Check sheet for the modelled part. Datum: model origin and axes. Units: mm. Face numbers are marked on the shaded views. A direction names the side the tool comes from. Round coordinates to 2 decimals unless told otherwise and drop trailing zeros. Order: outer loops, then holes, each group sorted by start corner. A loop starts at its lowest first (then second) coordinate and runs counter-clockwise, first axis right, second up. Notation, with made-up numbers: (24.5, 9) -> (73.5, 9) arc R28 cw to (73.5, 36) -> close; hole circle Ø9 at (24, 10.25). An arc over 180 degrees is marked (long way). Use CSV: the item, a comma, the result in double quotes.
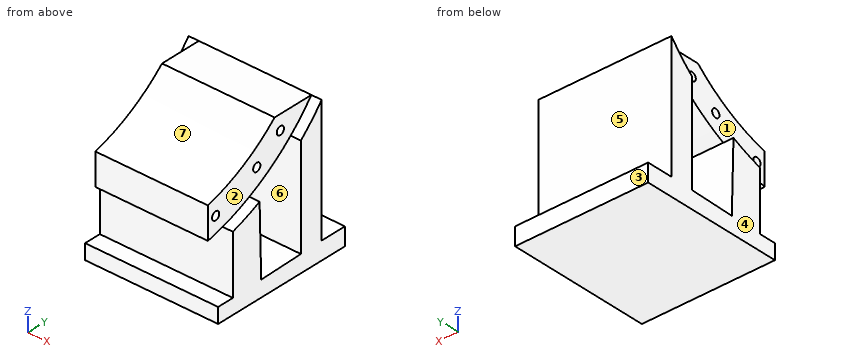
```python
from build123d import *

# Parameters (mm, degrees)
SKETCH1_W               = 130
SKETCH1_H               = 140
BOSS_EXTRUDE1_DEPTH     = 10
SKETCH14_W              = 130
SKETCH14_H              = 140
BOSS_EXTRUDE2_DEPTH     = 130
CUT_EXTRUDE2_DEPTH      = 299.998327755
CUT_EXTRUDE2_DEPTH_BACK = 299.998327755
SKETCH15_W              = 122.59192481
SKETCH15_H              = 25.689880701
CUT_EXTRUDE4_DEPTH      = 299.998327755
CUT_EXTRUDE4_DEPTH_BACK = 10
CUT_EXTRUDE5_DEPTH      = 10
CUT_EXTRUDE6_DEPTH      = 295.78805946
CUT_EXTRUDE6_DEPTH_BACK = 295.78805946
SKETCH19_R              = 4


with BuildPart() as part:
    # Sketch1 → Boss-Extrude1 (new body)
    with BuildSketch(Plane.XY):
        with Locations((65, 160)):
            Rectangle(SKETCH1_W, SKETCH1_H)
    extrude(amount=BOSS_EXTRUDE1_DEPTH)

    # Sketch14 → Boss-Extrude2 (add)
    with BuildSketch(Plane.XY.offset(10)):
        with Locations((65, 160)):
            Rectangle(SKETCH14_W, SKETCH14_H)
    extrude(amount=BOSS_EXTRUDE2_DEPTH)

    # Sketch15 → Cut-Extrude2 (cut, two sides: drawn at the far end of the back side and taken through both)
    with BuildSketch(Plane(origin=(130, 0, 0), x_dir=(0, 0, -1), z_dir=(1, 0, 0)).offset(-CUT_EXTRUDE2_DEPTH_BACK)):
        with BuildLine():
            Line((-140, 90), (-140, 163.652960017))
            ThreePointArc((-140, 163.652960017), (-114.94393992, 129.358801446), (-98.982103949, 90))
            Line((-98.982103949, 90), (-140, 90))
        make_face()
        with BuildLine():
            Line((-68.08230106, 90), (-14.839979069, 90))
            Line((-14.839979069, 90), (-14.839979069, 106.264255909))
            Line((-14.839979069, 106.264255909), (-72.486347105, 106.264255909))
            ThreePointArc((-72.486347105, 106.264255909), (-70.115745067, 98.177775893), (-68.08230106, 90))
        make_face()
        with Locations((-78.704037595, 217.15505965)):
            Rectangle(SKETCH15_W, SKETCH15_H)
        with BuildLine():
            Line((-16.807794328, 181.392341835), (-15.660073853, 137.574182571))
            Line((-15.660073853, 137.574182571), (-84.418578186, 135.773204516))
            ThreePointArc((-84.418578186, 135.773204516), (-98.429747838, 159.645053575), (-115.553810025, 181.392341835))
            Line((-115.553810025, 181.392341835), (-16.807794328, 181.392341835))
        make_face()
    extrude(amount=CUT_EXTRUDE2_DEPTH + CUT_EXTRUDE2_DEPTH_BACK, mode=Mode.SUBTRACT)

    # Sketch17 → Cut-Extrude4 (cut, two sides: drawn at the far end of the back side and taken through both)
    with BuildSketch(Plane(origin=(130, 0, 0), x_dir=(0, 0, -1), z_dir=(1, 0, 0)).offset(-CUT_EXTRUDE4_DEPTH_BACK)):
        with BuildLine():
            Line((-140, 204.310119299), (-140, 163.652960017))
            ThreePointArc((-140, 163.652960017), (-114.94393992, 129.358801446), (-98.982103949, 90))
            Line((-98.982103949, 90), (-68.08230106, 90))
            ThreePointArc((-68.08230106, 90), (-70.115745067, 98.177775893), (-72.486347105, 106.264255909))
            ThreePointArc((-72.486347105, 106.264255909), (-98.905883629, 160.339590918), (-140, 204.310119299))
        make_face()
    extrude(amount=CUT_EXTRUDE4_DEPTH + CUT_EXTRUDE4_DEPTH_BACK, mode=Mode.SUBTRACT)

    # Sketch18 → Cut-Extrude5 (cut)
    with BuildSketch(Plane.ZY):
        with BuildLine():
            Line((98.982103949, 90), (68.08230106, 90))
            ThreePointArc((68.08230106, 90), (94.271584258, 153.301538458), (140, 204.310119299))
            Line((140, 204.310119299), (140, 163.652960017))
            ThreePointArc((140, 163.652960017), (114.94393992, 129.358801446), (98.982103949, 90))
        make_face()
    extrude(amount=-CUT_EXTRUDE5_DEPTH, mode=Mode.SUBTRACT)

    # Sketch19 → Cut-Extrude6 (cut, two sides: drawn at the far end of the back side and taken through both)
    with BuildSketch(Plane.ZY.offset(-10).offset(-CUT_EXTRUDE6_DEPTH_BACK)):
        with Locations((85.807813583, 98.537572545)):
            Circle(SKETCH19_R)
        with Locations((106.132515119, 143.973580916)):
            Circle(SKETCH19_R)
        with Locations((125.519269901, 170.036489259)):
            Circle(SKETCH19_R)
    extrude(amount=CUT_EXTRUDE6_DEPTH + CUT_EXTRUDE6_DEPTH_BACK, mode=Mode.SUBTRACT)


solid = part.part
```
Q1. Access from +Z, -Z, +X, -X, +Y, -Y to the whole of each face (thin tool, end or side, straight path). Record for the marked faces 1, 2 and 3.
Result sheet:
face 1,"+Z, -X, -Y"
face 2,"+Z, +X, -Y"
face 3,"+Z, -Z, +X, -X, +Y"
Q2. Sectioned sample at C-C, the plane y = 178. Enter the section's corners in (x, z).
Result sheet:
outline,"(0, 0) -> (130, 0) -> (130, 16.72) -> (0, 16.72) -> close; (10, 112.55) -> (120, 112.55) -> (120, 140) -> (10, 140) -> close"
Q3. Mould release check, pull along Y, two halves, no side actions. Record for the marked faces 4, 5, 6 and 7: pulls with the +Y half, pulls with the -Y half, needs draft (parallel to the pull), parting line crosses it, or undercut.
Result sheet:
face 4,"needs draft"
face 5,"pulls with the +Y half"
face 6,"undercut"
face 7,"pulls with the -Y half"
Q4. Sectioned sample at A-A, the plane z = 63.5. Enter the section's corners in (x, y), then the cut area to 3 significant figures.
Result sheet:
outline,"(0, 106.26) -> (130, 106.26) -> (130, 136.32) -> (0, 136.32) -> close; (0, 181.39) -> (130, 181.39) -> (130, 204.31) -> (0, 204.31) -> close"
area,"6,890 mm^2"
Q5. Sectioned sample at D-D, the plane y = 123. Enter the section's corners in (x, z), then the cut area to 3 significant figures.
Result sheet:
outline,"(0, 0) -> (130, 0) -> (130, 78.59) -> (120, 78.59) -> (120, 111.57) -> (10, 111.57) -> (10, 78.59) -> (0, 78.59) -> close"
area,"13,800 mm^2"
Q6. Go/stop test with flat-tipped pins: pin 1 (1.5 mm diameter, centred on x = 55, z = 33.5, fed in from -Y); pin 2 (1.5 mm diameter, centred on x = 107, z = 60, fed in from +Y); pin 3 (5 mm diameter, centred on y = 143.97, z = 106.13, fed in from +X); pin 4 (1 mm diameter, centred on x = 60.5, y = 127, fed in from +Z). Record where each tip stops, or that it passes through.
Result sheet:
pin 1,"stops at y = 106.26"
pin 2,"stops at y = 204.31"
pin 3,"passes through"
pin 4,"stops at z = 113.92"
Q7. Sectioned sample at B-B, the plane x = 34. Enter the section's corners in (y, z).
Result sheet:
outline,"(90, 0) -> (230, 0) -> (230, 17.41) -> (204.31, 17.41) -> (204.31, 140) -> (163.65, 140) arc R173.29 cw to (90, 98.98) -> (90, 68.08) arc R203.29 ccw to (106.26, 72.49) -> (106.26, 14.84) -> (90, 14.84) -> close; hole circle Ø8 at (98.54, 85.81); hole (135.77, 84.42) -> (137.57, 15.66) -> (181.39, 16.81) -> (181.39, 115.55) arc R203.29 cw to start; hole circle Ø8 at (143.97, 106.13); hole circle Ø8 at (170.04, 125.52)"
Q8. Scan lines: L1, parallel to Z at x = 112, y = 101; L2, parallel to Z at x = 75, y = 139; L3, parallel to Z at x = 72, y = 174.5. Record each from-to range of solid material in increasing order.
Result sheet:
L1,"z = 0 to 14.84, 70.9 to 82.66, 88.96 to 102.33"
L2,"z = 0 to 15.7, 86.06 to 120.73"
L3,"z = 0 to 16.63, 109.6 to 140"
